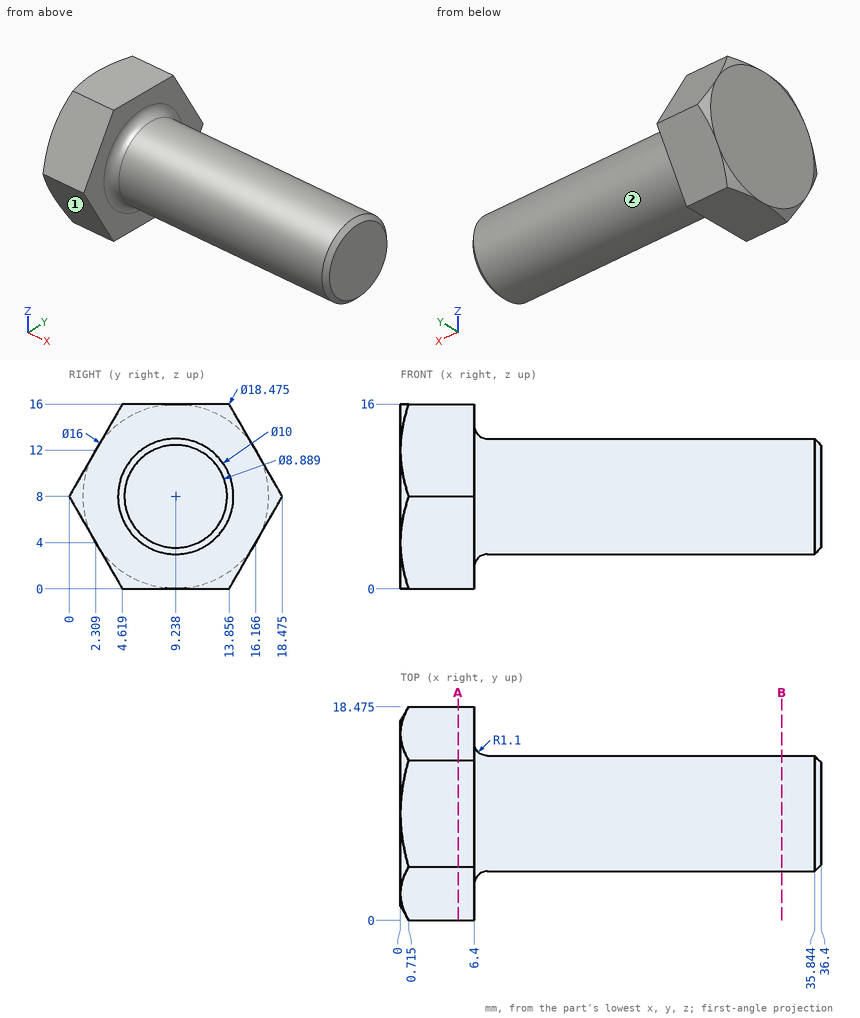
Geometry check sheet. Reference: drawing and pictorial views, mm from the part's lowest x, y, z. A direction names the side the tool comes from. Coordinates: 2 decimals unless noted, no trailing zeros. Order: outer loops, then holes, each group sorted by start corner. A loop starts at its lowest first (then second) coordinate and runs counter-clockwise, first axis right, second up. Notation, with made-up numbers: (-29, -27.5) - (-10, -27.5) arc R33 cw to (-10, 4.5) - close; hole circle Ø7 at (-14, -11.75). An arc over 180 degrees is marked (long way). One line per item, written item: value.
(1) Access from +Z, -Z, +X, -X, +Y, -Y to the whole of each face (thin tool, end or side, straight path). Record for the marked faces 1 and 2.
Data:
face 1: -Z, +X, -X, -Y
face 2: +X
(2) Sectioned sample at A-A (x = 5). Enter the section's corners in (y, z) (1 decimal), and give its area (3 significant figures).
Data:
outline: (0, 8) - (4.6, 0) - (13.9, 0) - (18.5, 8) - (13.9, 16) - (4.6, 16) - close
area: 222 mm^2
(3) Depth check by flat-ended pin: pin 1 Ø2 at (x, z) = (24, 4.5) entering from +Y; pin 2 Ø3 at (x, y) = (31.5, 4.5) entering from -Z; pin 3 Ø4 at (x, z) = (32, 4.5) entering from -Y. Enter the tip coordinate at first touch or a pass-through.
Data:
pin 1: stops at y = 13.57
pin 2: stops at z = 4.19
pin 3: stops at y = 4.47
(4) Sectioned sample at B-B (x = 33). Enter the section's corners in (y, z).
Data:
outline: circle Ø10 at (9.24, 8)
(5) Thickness scan on probe 1 along X at (y, z) = (16, 11.5); probe 2 along Z at (x, y) = (22.5, 9.5); probe 3 along Z at (x, y) = (27.5, 6.25). Record the ranges inside material, lowest first. Write a range as from..to.
Data:
probe 1: x = 0..6.4
probe 2: z = 3.01..12.99
probe 3: z = 3.99..12.01
